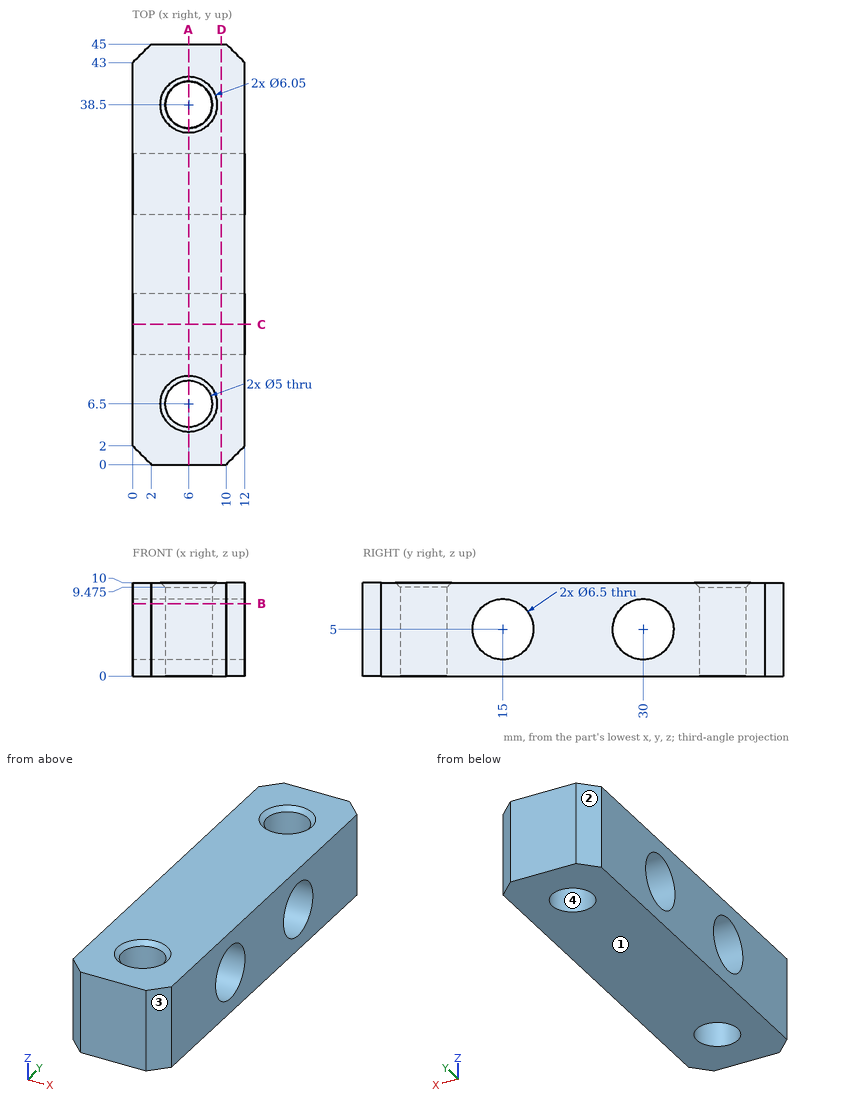
Check sheet for the drawn part. Datum: minimum x, y, z corner. Units: mm. Round coordinates to 2 decimals unless told otherwise and drop trailing zeros. Write each loop counter-clockwise with the first axis right and the second up, starting at its lowest first coordinate (ties: lowest second). Pieces come first, ordered by that corner, then holes. Notation, with made-up numbers: (69, -40) -> (96, -40) arc R10 cw to (96, -31) -> close; hole circle Ø5 at (83, -17). An arc over 180 degrees is marked (long way). Write each question's results on one line, items separated by ' | '.
Q1. Go/stop test with flat-tipped pins: pin 1 Ø5 at (y, z) = (15, 5) entering from +X; pin 2 Ø5 at (y, z) = (12, 5) entering from +X. Record where each tip stops, or that it passes through.
Derived:
pin 1: passes through | pin 2: stops at x = 12
Q2. Sectioned sample at D-D, the plane x = 9.5. Record the boundary of the cut face in (y, z), and give its area (3 significant figures).
Derived:
outline: (0, 0) -> (45, 0) -> (45, 10) -> (0, 10) -> close; hole circle Ø6.5 at (15, 5); hole circle Ø6.5 at (30, 5) | area: 384 mm²
Q3. Draft check along Y on the marked faces 1, 2, 3 and 4. Enter one of: released by +Y, released by -Y, zero draft, split by the parting line, or undercut.
Derived:
face 1: zero draft | face 2: released by +Y | face 3: released by -Y | face 4: undercut
Q4. Sectioned sample at B-B, the plane z = 7.75. Record the boundary of the cut face in (x, y), and give its area (3 significant figures).
Derived:
outline: (0, 2) -> (2, 0) -> (10, 0) -> (12, 2) -> (12, 13.27) -> (0, 13.27) -> close; (0, 16.73) -> (12, 16.73) -> (12, 28.27) -> (0, 28.27) -> close; (0, 31.73) -> (12, 31.73) -> (12, 43) -> (10, 45) -> (2, 45) -> (0, 43) -> close; hole circle Ø5 at (6, 6.5); hole circle Ø5 at (6, 38.5) | area: 410 mm²
Q5. Thickness scan on probe 1 along Y at (x, z) = (6, 6.5); probe 2 along Y at (x, z) = (7, 5); probe 3 along Y at (x, z) = (10.5, 7.25). Record the ranges inside material, lowest first.
Derived:
probe 1: y = 0 to 4, 9 to 12.12, 17.88 to 27.12, 32.88 to 36, 41 to 45 | probe 2: y = 0 to 4.21, 8.79 to 11.75, 18.25 to 26.75, 33.25 to 36.21, 40.79 to 45 | probe 3: y = 0.5 to 12.65, 17.35 to 27.65, 32.35 to 44.5
Q6. Sectioned sample at A-A, the plane x = 6. Record the boundary of the cut face in (y, z) (3 decimals).
Derived:
outline: (0, 0) -> (4, 0) -> (4, 9.475) -> (3.475, 10) -> (0, 10) -> close; (9, 0) -> (36, 0) -> (36, 9.475) -> (35.475, 10) -> (9.525, 10) -> (9, 9.475) -> close; (41, 0) -> (45, 0) -> (45, 10) -> (41.525, 10) -> (41, 9.475) -> close; hole circle Ø6.5 at (15, 5); hole circle Ø6.5 at (30, 5)
Q7. Sectioned sample at C-C, the plane y = 15. Record the boundary of the cut face in (x, z), and give its area (3 significant figures).
Derived:
outline: (0, 0) -> (12, 0) -> (12, 1.75) -> (0, 1.75) -> close; (0, 8.25) -> (12, 8.25) -> (12, 10) -> (0, 10) -> close | area: 42.0 mm²
